The figure shows three views and two pictorial views of one solid part (mm, origin at its lowest corner). Answer the questions. A direction names the side the tool comes from. Give positions to 0.01 mm unless a question says otherwise; leave off trailing zeros. Order: outer loops, then holes, each group sorted by start corner. A loop starts at its lowest first (then second) coordinate and runs counter-clockwise, first axis right, second up. Notation, with made-up numbers: (18.25, -14.5) - (76.25, -14.5) arc R25 ccw to (76.25, 11.5) - close; hole circle Ø1 at (54.5, 73.25). An arc over 180 degrees is marked (long way). Answer as a JSON object with one key per item and string values. Group by question number.
Q1. Consider line 1 (X direction, y = 73, z = 44); line 2 (Z direction, x = 66, y = 4.5); line 3 (Z direction, x = 54, y = 39). Determine where each line is inside the solid, lowest interval first.
Q2. Given pin 1 (8 mm diameter, centred on x = 87.5, z = 81.5, fed in from +Y); pin 2 (3.5 mm diameter, centred on x = 75.5, y = 7, fed in from +Z); pin 3 (1.5 mm diameter, centred on x = 92, y = 44, fed in from +Z), each flat-ended and moving along its own axis, determine where each tip first touches the part or whether it passes through.
Q3. A cutting plane is placed at C-C, the plane x = 24. Give the vertices of the cut face in (y, z).
Q4. For the marked faces 1, 2 and 3, determine the directions among +Z, -Z, +X, -X, +Y, -Y from which every point of the face is accessible in a straight line to the end or side of a thin tool.
Q5. The mould has two halves that part along Z. Classify the marked faces 4, 5, 6 and 7: released by +Z, released by -Z, zero draft, split by the parting line, or undercut.
Q6. A cutting plane is placed at B-B, the plane z = 93.5. Give the vertices of the cut face in (x, y).
Q7. A cutting plane is placed at D-D, the plane z = 62. Give the vertices of the cut face in (x, y).
Q8. A cutting plane is placed at A-A, the plane y = 59. Give the vertices of the cut face in (x, z).
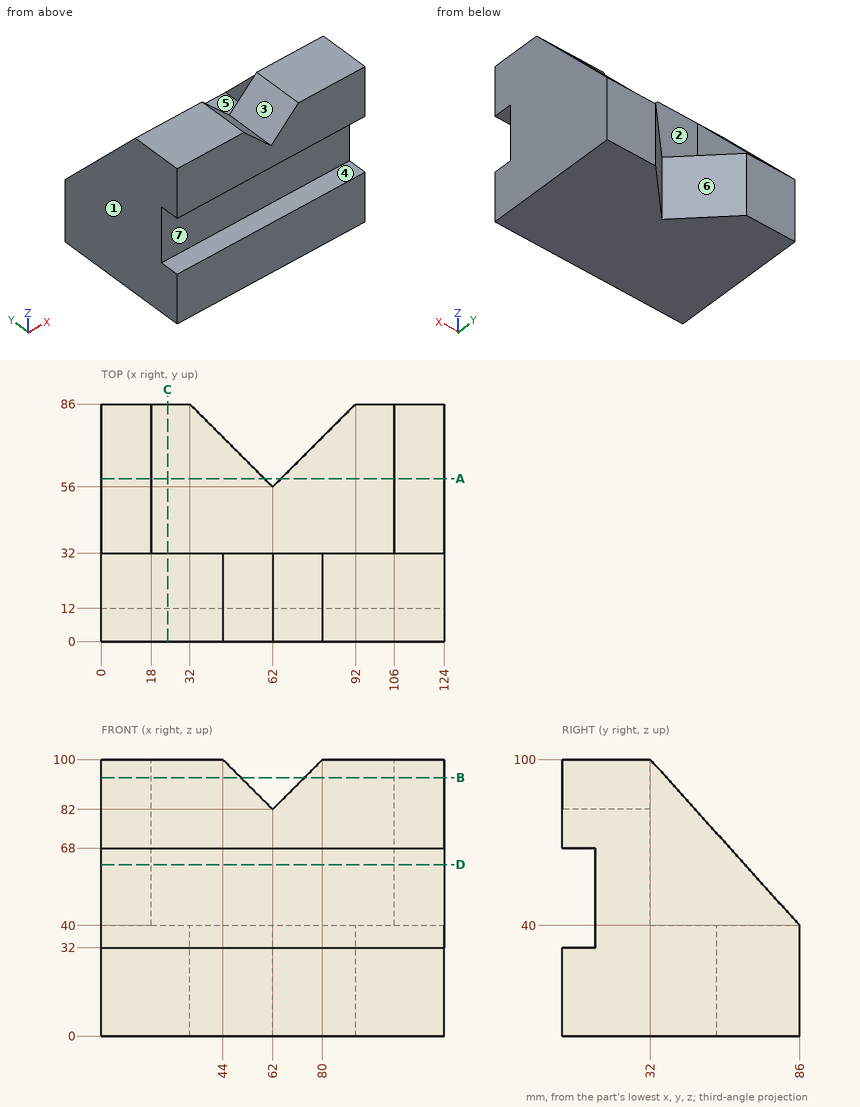
Reply:
{
 "1": {"line 1": "x = 0 to 18, 106 to 124", "line 2": "z = 0 to 32, 68 to 86", "line 3": "z = 0 to 40"},
 "2": {"pin 1": "stops at y = 32", "pin 2": "stops at z = 97.25", "pin 3": "stops at z = 40"},
 "3": {"outline": "(0, 0) - (86, 0) - (86, 40) - (32, 40) - (32, 100) - (0, 100) - (0, 68) - (12, 68) - (12, 32) - (0, 32) - close"},
 "4": {"face 1": "+Z, -Z, -X, +Y, -Y", "face 2": "+Z, +Y", "face 3": "+Z, +Y, -Y"},
 "5": {"face 4": "undercut", "face 5": "released by +Z", "face 6": "zero draft", "face 7": "undercut"},
 "6": {"outline": "(0, 0) - (50.5, 0) - (50.5, 32) - (18, 32) - (18, 37.85) - (0, 37.85) - close; (73.5, 0) - (124, 0) - (124, 37.85) - (106, 37.85) - (106, 32) - (73.5, 32) - close"},
 "7": {"outline": "(0, 12) - (124, 12) - (124, 66.2) - (106, 66.2) - (106, 32) - (18, 32) - (18, 66.2) - (0, 66.2) - close"},
 "8": {"outline": "(0, 0) - (59, 0) - (59, 40) - (18, 40) - (18, 70) - (0, 70) - close; (65, 0) - (124, 0) - (124, 70) - (106, 70) - (106, 40) - (65, 40) - close"}
}
